Here's how the part is built. I have some questions about the finished solid (model axes, mm). Face numbers are marked on the shaded views. A direction names the side the tool comes from. Round coordinates to 2 decimals unless told otherwise and drop trailing zeros. Loops run counter-clockwise (first coordinate to the right, second up) from the corner with the lowest first, then second, coordinate; pieces in that order, holes last. Notation, with made-up numbers: M 78.5,-34.75 L 120.5,-34.75 A21 ccw 120.5,-11.75 Z; hole C 34,28 d11. An arc over 180 degrees is marked long. Use a Markdown table: item, result.
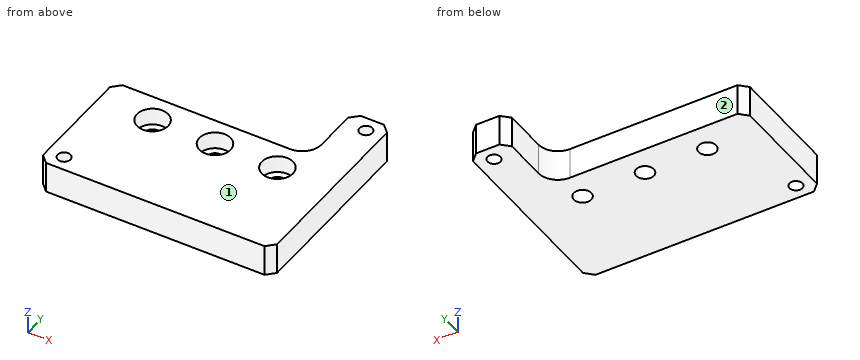
from build123d import *

# Parameters (mm, degrees)
SKETCH1_W                                           = 60
SKETCH1_H                                           = 50
BOSS_EXTRUDE1_DEPTH                                 = 8
CBORE_FOR_M4_HEX_SOCKET_HEAD_CAP_SCREW1_D           = 4.5
CBORE_FOR_M4_HEX_SOCKET_HEAD_CAP_SCREW1_CBORE_D     = 8
CBORE_FOR_M4_HEX_SOCKET_HEAD_CAP_SCREW1_CBORE_DEPTH = 4.4
M4_TAPPED_HOLE1_D                                   = 3.3
CHAMFER1_SIZE                                       = 2
SKETCH6_W                                           = 50
SKETCH6_H                                           = 18
CUT_EXTRUDE1_DEPTH                                  = 79.511145706
CHAMFER2_SIZE                                       = 2
FILLET1_R                                           = 5


with BuildPart() as part:
    # Sketch1 → Boss-Extrude1 (new body)
    with BuildSketch(Plane.XY):
        with Locations((30, 25)):
            Rectangle(SKETCH1_W, SKETCH1_H)
    extrude(amount=BOSS_EXTRUDE1_DEPTH)

    # CBORE for M4 Hex Socket Head Cap Screw1 (through all)
    with Locations(Plane.XY.offset(8)):
        with Locations((46, 25), (30, 25), (14, 25)):
            CounterBoreHole(CBORE_FOR_M4_HEX_SOCKET_HEAD_CAP_SCREW1_D / 2, CBORE_FOR_M4_HEX_SOCKET_HEAD_CAP_SCREW1_CBORE_D / 2, CBORE_FOR_M4_HEX_SOCKET_HEAD_CAP_SCREW1_CBORE_DEPTH)

    # M4 Tapped Hole1 (through all)
    with Locations(Plane.XY.offset(8)):
        with Locations((55.7, 46.2), (4.3, 3.8)):
            Hole(M4_TAPPED_HOLE1_D / 2)

    # Chamfer1
    chamfer1_edges = [part.edges().sort_by_distance(p)[0] for p in [
        (0, 50, 4),
        (60, 50, 4),
        (60, 0, 4),
        (0, 0, 4),
    ]]
    chamfer(chamfer1_edges, length=CHAMFER1_SIZE)

    # Sketch6 → Cut-Extrude1 (cut, through all)
    with BuildSketch(Plane(origin=(0, 0, 0), x_dir=(-1, 0, 0), z_dir=(0, 0, -1))):
        with Locations((-25, 41)):
            Rectangle(SKETCH6_W, SKETCH6_H)
    extrude(amount=-CUT_EXTRUDE1_DEPTH, mode=Mode.SUBTRACT)

    # Chamfer2
    chamfer2_edges = [part.edges().sort_by_distance(p)[0] for p in [
        (50, 50, 4),
        (0, 32, 4),
    ]]
    chamfer(chamfer2_edges, length=CHAMFER2_SIZE)

    # Fillet1
    fillet1_edges = [part.edges().sort_by_distance(p)[0] for p in [
        (50, 32, 4),
    ]]
    fillet(fillet1_edges, radius=FILLET1_R)


solid = part.part
1. Imagine slicing it at A-A, the plane y = 46.2. Write out the boundary of the cut face in (x, z), then the cut area to 3 significant figures.
Answer sheet:
| item | result |
|---|---|
| outline | M 50,0 L 54.05,0 L 54.05,8 L 50,8 Z; M 57.35,0 L 60,0 L 60,8 L 57.35,8 Z |
| area | 53.6 mm2 |
2. Which directions (+Z, -Z, +X, -X, +Y, -Y) give clear straight access to the entire face, cutting with the end or side of a thin tool? Please do the marked faces 1 and 2.
Answer sheet:
| item | result |
|---|---|
| face 1 | +Z, +X, -X, +Y, -Y |
| face 2 | +Z, -Z, -X, +Y |
3. For pin 1 Ø7 at (x, y) = (30, 25) entering from +Z; pin 2 Ø1.5 at (x, z) = (40, 5.5) entering from +Y; pin 3 Ø4 at (y, z) = (41.5, 5.5) entering from -X, each with a flat end and sliding along its axis, tell me the tip position at first contact or that it passes through.
Answer sheet:
| item | result |
|---|---|
| pin 1 | z = 3.6 |
| pin 2 | y = 32 |
| pin 3 | x = 50 |
4. I need wall thicknesses on probe 1 along X at (y, z) = (27, 4); probe 2 along Y at (x, z) = (4.5, 7.5); probe 3 along Y at (x, z) = (14, 2.35). Which ranges of each line are inside material? Lowest first, please. Write a range as from..to.
Answer sheet:
| item | result |
|---|---|
| probe 1 | 0..10.54, 17.46..26.54, 33.46..42.54, 49.46..60 |
| probe 2 | 0..2.16, 5.44..32 |
| probe 3 | 0..22.75, 27.25..32 |
5. Imagine slicing it at C-C, the plane y = 25. Write out the boundary of the cut face in (x, z).
Answer sheet:
| item | result |
|---|---|
| outline | M 0,0 L 11.75,0 L 11.75,3.6 L 10,3.6 L 10,8 L 0,8 Z; M 16.25,0 L 27.75,0 L 27.75,3.6 L 26,3.6 L 26,8 L 18,8 L 18,3.6 L 16.25,3.6 Z; M 32.25,0 L 43.75,0 L 43.75,3.6 L 42,3.6 L 42,8 L 34,8 L 34,3.6 L 32.25,3.6 Z; M 48.25,0 L 60,0 L 60,8 L 50,8 L 50,3.6 L 48.25,3.6 Z |
6. Imagine slicing it at B-B, the plane x = 4.3. Write out the boundary of the cut face in (y, z), then the cut area to 3 significant figures.
Answer sheet:
| item | result |
|---|---|
| outline | M 0,0 L 2.15,0 L 2.15,8 L 0,8 Z; M 5.45,0 L 32,0 L 32,8 L 5.45,8 Z |
| area | 230 mm2 |
7. Imagine slicing it at D-D, the plane z = 1.75. Write out the boundary of the cut face in (x, y).
Answer sheet:
| item | result |
|---|---|
| outline | M 0,2 L 2,0 L 58,0 L 60,2 L 60,48 L 58,50 L 52,50 L 50,48 L 50,37 A5 cw 45,32 L 2,32 L 0,30 Z; hole C 4.3,3.8 d3.3; hole C 14,25 d4.5; hole C 30,25 d4.5; hole C 46,25 d4.5; hole C 55.7,46.2 d3.3 |
